Verification items for this drawing (mm, ordinates from the low corner). A direction names the side the tool comes from. Round coordinates to 2 decimals unless told otherwise and drop trailing zeros. Loops run counter-clockwise (first coordinate to the right, second up) from the corner with the lowest first, then second, coordinate; pieces in that order, holes last. Notation, with made-up numbers: (82, -12.5) - (136, -12.5) arc R20 ccw to (136, 19.5) - close; hole circle Ø3 at (71, 19). An arc over 180 degrees is marked (long way). Answer in a Markdown table with one row per item. Add a question column.
(1) Cross-section at C-C on y = 146.5. Enter the section's corners in (x, z), then the cut area to 3 significant figures.
(2) Access from +Z, -Z, +X, -X, +Y, -Y to the whole of each face (thin tool, end or side, straight path). Record for the marked faces 1 and 2.
(3) Thickness scan on line 1 along Y through (x, z) = (53, 5.75); line 2 along X through (y, z) = (146.5, 9.75); line 3 along X through (y, z) = (170.5, 6.5). Record the ranges inside material, lowest first.
(4) Gauge pin test, flat ends, axial feed: pin 1 (1 mm diameter, centred on x = 30, z = 3, fed in from +Y); pin 2 (2 mm diameter, centred on y = 32, z = 10, fed in from -X); pin 3 (8 mm diameter, centred on x = 8, z = 7, fed in from -Y). Record the tip position at first contact, or that the pin passes through.
(5) Cross-section at A-A on z = 7. Enter the section's corners in (x, y), then the cut area to 3 significant figures.
(6) Cross-section at D-D on x = 35.5. Enter the section's corners in (y, z), then the cut area to 3 significant figures.
(7) Cross-section at B-B on x = 53. Enter the section's corners in (y, z), then the cut area to 3 significant figures.
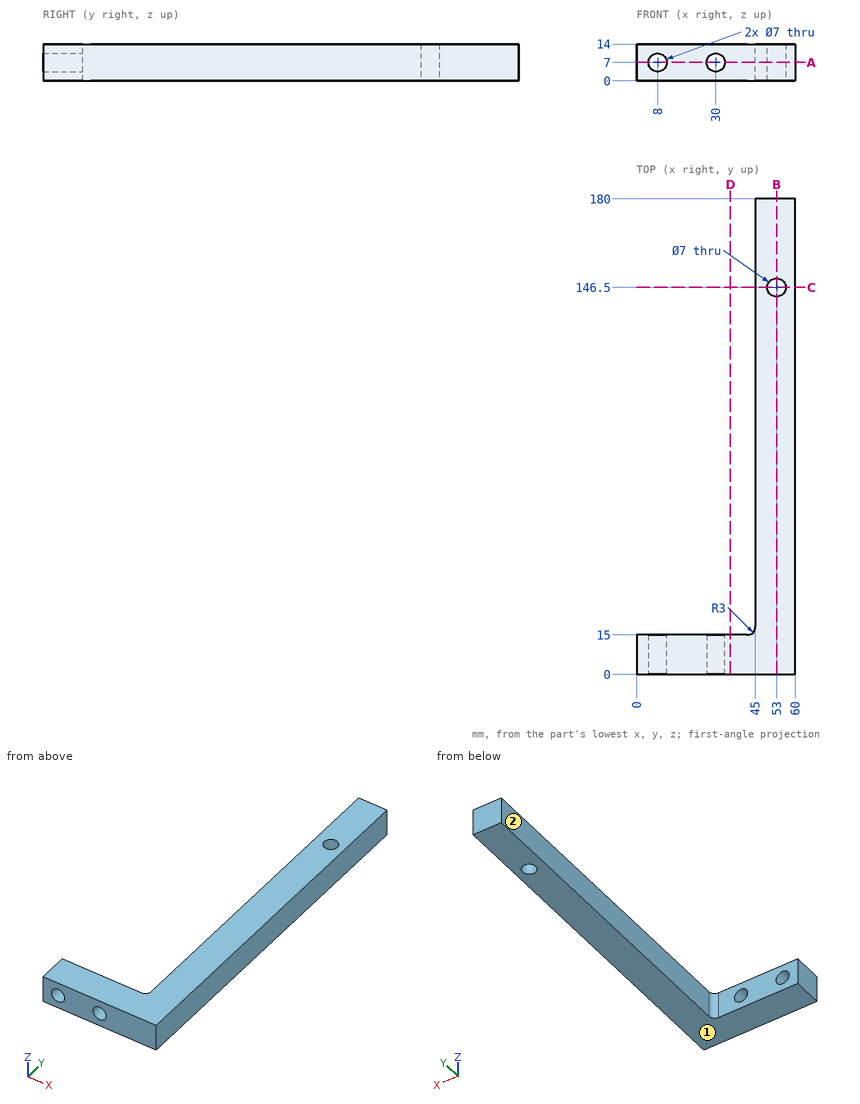
Answers:
| question | item | result |
|---|---|---|
| 1 | outline | (45, 0) - (49.5, 0) - (49.5, 14) - (45, 14) - close; (56.5, 0) - (60, 0) - (60, 14) - (56.5, 14) - close |
| 1 | area | 112 mm^2 |
| 2 | face 1 | -Z, +X, -X, +Y, -Y |
| 2 | face 2 | +Z, -Z, -X, +Y |
| 3 | line 1 | y = 0 to 143, 150 to 180 |
| 3 | line 2 | x = 45 to 49.5, 56.5 to 60 |
| 3 | line 3 | x = 45 to 60 |
| 4 | pin 1 | stops at y = 15 |
| 4 | pin 2 | stops at x = 45 |
| 4 | pin 3 | stops at y = 0 |
| 5 | outline | (0, 0) - (4.5, 0) - (4.5, 15) - (0, 15) - close; (11.5, 0) - (26.5, 0) - (26.5, 15) - (11.5, 15) - close; (33.5, 0) - (60, 0) - (60, 180) - (45, 180) - (45, 18) arc R3 cw to (42, 15) - (33.5, 15) - close; hole circle Ø7 at (53, 146.5) |
| 5 | area | 3,130 mm^2 |
| 6 | outline | (0, 0) - (15, 0) - (15, 14) - (0, 14) - close |
| 6 | area | 210 mm^2 |
| 7 | outline | (0, 0) - (143, 0) - (143, 14) - (0, 14) - close; (150, 0) - (180, 0) - (180, 14) - (150, 14) - close |
| 7 | area | 2,420 mm^2 |
